Source: three-view drawing plus pictorial views. Frame: mm from the lowest corner of the part. A direction names the side the tool comes from. Round coordinates to 2 decimals unless told otherwise and drop trailing zeros. Order: outer loops, then holes, each group sorted by start corner. A loop starts at its lowest first (then second) coordinate and runs counter-clockwise, first axis right, second up. Notation, with made-up numbers: (70, -27) -> (81, -27) arc R26 cw to (81, -7) -> close; hole circle Ø5 at (13.5, 47). An arc over 180 degrees is marked (long way). Answer as CSV lines item,"result".
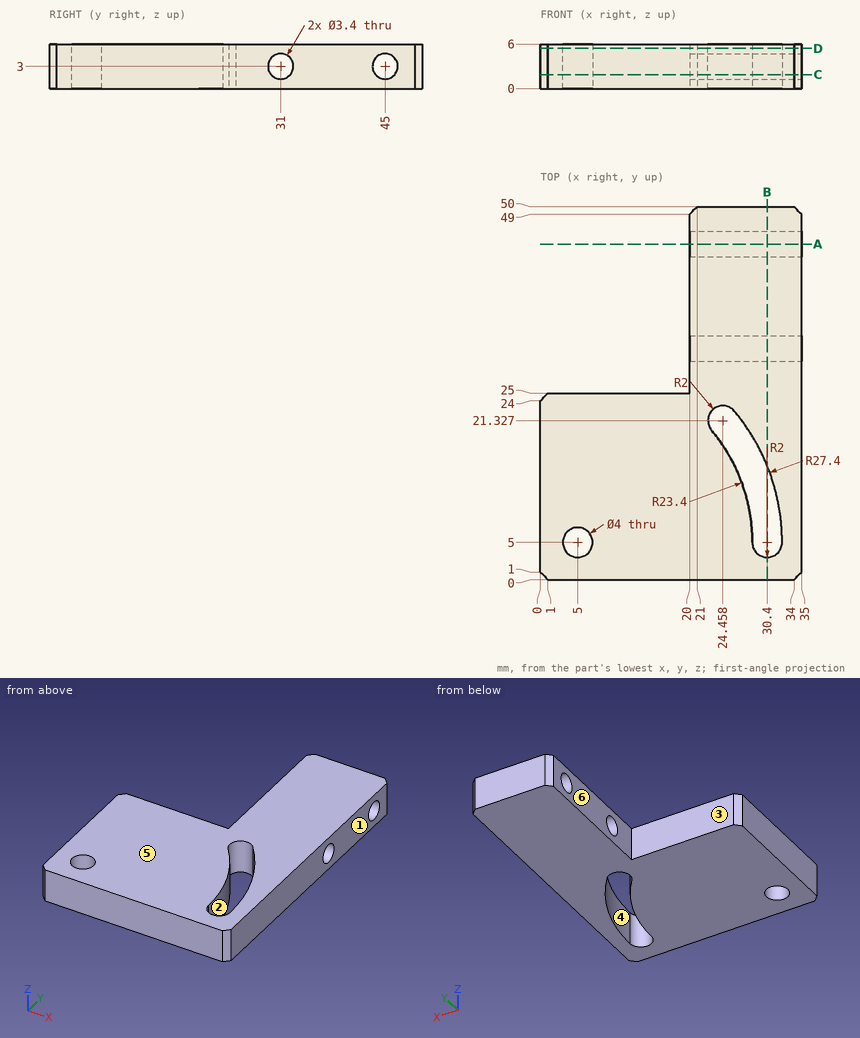
1. Section query A-A on y = 45. Return loops of the section in (x, z).
Results below:
outline,"(20, 0) -> (35, 0) -> (35, 1.3) -> (20, 1.3) -> close; (20, 4.7) -> (35, 4.7) -> (35, 6) -> (20, 6) -> close"
2. Mould query, pull axis X, two halves, no side actions, for the marked faces 4, 5 and 6. Classes: released by +X, released by -X, zero draft, split by the parting line, or undercut.
Results below:
face 4,"undercut"
face 5,"zero draft"
face 6,"released by -X"
3. Line query: L1, parallel to Y at x = 5, z = 3.6; L2, parallel to Y at x = 29.75, z = 3 (1 decimal); L3, parallel to Y at x = 11.5, z = 0.3. Output: solid intervals per line, ascending. Write a range as [from, to].
Results below:
L1,"[0, 3], [7, 25]"
L2,"[0, 3.1], [16.8, 29.3], [32.7, 43.3], [46.7, 50]"
L3,"[0, 25]"
4. Section query C-C on z = 1.9. Return loops of the section in (x, y) (1 decimal), and give its area (3 significant figures).
Results below:
outline,"(0, 1) -> (1, 0) -> (34, 0) -> (35, 1) -> (35, 29.7) -> (20, 29.7) -> (20, 25) -> (1, 25) -> (0, 24) -> close; (20, 32.3) -> (35, 32.3) -> (35, 43.7) -> (20, 43.7) -> close; (20, 46.3) -> (35, 46.3) -> (35, 49) -> (34, 50) -> (21, 50) -> (20, 49) -> close; hole circle Ø4 at (5, 5); hole (22.9, 20) arc R23.4 cw to (28.4, 5) arc R2 ccw to (32.4, 5) arc R27.4 ccw to (26, 22.6) arc R2 ccw to start"
area,"1,070 mm2"
5. Reachability of the marked faces 1, 2 and 3 from +Z, -Z, +X, -X, +Y, -Y: full face, straight path, thin tool, end or side. Return the list, or none.
Results below:
face 1,"+Z, -Z, +X, +Y, -Y"
face 2,"+Z, -Z"
face 3,"+Z, -Z, -X, +Y"
6. Section query B-B on x = 30.4. Return loops of the section in (y, z), and give its area (3 significant figures).
Results below:
outline,"(0, 0) -> (3, 0) -> (3, 6) -> (0, 6) -> close; (15.28, 0) -> (50, 0) -> (50, 6) -> (15.28, 6) -> close; hole circle Ø3.4 at (31, 3); hole circle Ø3.4 at (45, 3)"
area,"208 mm2"
7. Section query D-D on z = 5.4. Return loops of the section in (x, y) (1 decimal).
Results below:
outline,"(0, 1) -> (1, 0) -> (34, 0) -> (35, 1) -> (35, 49) -> (34, 50) -> (21, 50) -> (20, 49) -> (20, 25) -> (1, 25) -> (0, 24) -> close; hole circle Ø4 at (5, 5); hole (22.9, 20) arc R23.4 cw to (28.4, 5) arc R2 ccw to (32.4, 5) arc R27.4 ccw to (26, 22.6) arc R2 ccw to start"
8. Pin query (flat end, axial travel): pin 1 (5 mm diameter, centred on x = 5, y = 5, fed in from -Z); pin 2 (3 mm diameter, centred on x = 10.5, z = 3.5, fed in from +Y). Return the tip coordinate at first contact, or that it passes through.
Results below:
pin 1,"z = 0"
pin 2,"y = 25"
